```python
from build123d import *

# Parameters (mm, degrees)
SKETCH_1_W          = 48
SKETCH_1_H          = 30
EXTRUDE_1_DEPTH     = 30
SKETCH_2_W          = 28
SKETCH_2_H          = 15
CUT_EXTRUDE_1_DEPTH = 20
SKETCH_3_R          = 2.2
CUT_EXTRUDE_2_DEPTH = 20
SKETCH_4_R          = 2.5
CUT_EXTRUDE_3_DEPTH = 30
CUT_EXTRUDE_START   = -30
SKETCH_8_W          = 48
SKETCH_8_H          = 7
CUT_EXTRUDE_5_DEPTH = 30


with BuildPart() as part:
    # 草图1 → 凸台-拉伸1 (new body)
    with BuildSketch(Plane.XY):
        with Locations((-0.545454545, 1.527272727)):
            Rectangle(SKETCH_1_W, SKETCH_1_H)
    extrude(amount=EXTRUDE_1_DEPTH)

    # 草图2 → 切除-拉伸1 (cut)
    with BuildSketch(Plane(origin=(0, 0, 0), x_dir=(-1, 0, 0), z_dir=(0, 0, -1))):
        with Locations((0.545454545, -5.972727273)):
            Rectangle(SKETCH_2_W, SKETCH_2_H)
    extrude(amount=-CUT_EXTRUDE_1_DEPTH, mode=Mode.SUBTRACT)

    # 草图3 → 切除-拉伸2 (cut)
    with BuildSketch(Plane(origin=(0, 0, 20), x_dir=(-1, 0, 0), z_dir=(0, 0, -1))):
        with Locations((-10.454545455, -3.472727273)):
            Circle(SKETCH_3_R)
        with Locations((11.545454545, -3.472727273)):
            Circle(SKETCH_3_R)
    extrude(amount=-CUT_EXTRUDE_2_DEPTH, mode=Mode.SUBTRACT)

    # 草图4 → 切除-拉伸3 (cut)
    with BuildSketch(Plane.XZ.offset(13.472727273)):
        with Locations(Location((-19.545454545, 5, 0), (0, 0, 270))):
            Circle(SKETCH_4_R)
        with Locations(Location((-19.545454545, 23, 0), (0, 0, 270))):
            Circle(SKETCH_4_R)
        with Locations(Location((18.454545455, 23, 0), (0, 0, 270))):
            Circle(SKETCH_4_R)
        with Locations(Location((18.454545455, 5, 0), (0, 0, 270))):
            Circle(SKETCH_4_R)
    extrude(amount=-CUT_EXTRUDE_3_DEPTH, mode=Mode.SUBTRACT)

    # 草图8 → 切除-拉伸5 (cut)
    with BuildSketch(Plane.XY.offset(30).offset(CUT_EXTRUDE_START)):
        with Locations((-0.545454545, 13.027272727)):
            Rectangle(SKETCH_8_W, SKETCH_8_H)
    extrude(amount=CUT_EXTRUDE_5_DEPTH, mode=Mode.SUBTRACT)


solid = part.part
```
The listing builds one solid part. Answer for the finished solid, in the listing's coordinates (mm). A direction names the side the tool comes from. Round coordinates to 2 decimals unless told otherwise and drop trailing zeros. Write each loop counter-clockwise with the first axis right and the second up, starting at its lowest first coordinate (ties: lowest second). Pieces come first, ordered by that corner, then holes. Notation, with made-up numbers: (49.5, 19) -> (96.5, 19) arc R28 ccw to (96.5, 42) -> close; hole circle Ø2 at (-40, 85). An arc over 180 degrees is marked (long way). Answer as a JSON object with one key per item and string values. Group by question number.
Q1. Determine the mould class of faces 1 (the face through (-21.07, -2.13, 24.98)), 2 (the face through (-14.545, -6, 10)), 3 (the face through (-1, 3, 0)), 4 (the face through (-1, -2, 30)) for opening direction Z: pulls with the +Z half, pulls with the -Z half, needs draft (parallel to the pull), parting line crosses it, or undercut.
Q2. Which of the six approach directions +Z, -Z, +X, -X, +Y, -Y give full straight-line access (tool end or side, diameter ignored) to faces 5 (the face through (-21.763, -2.134, 3.846)), 6 (the face through (0, 1.527, 10))?
Q3. Section B-B (z = 24.75) is taken. Write down the section's boundary in (x, y).
Q4. Straight lines are drawn through the part: line 1 along X through (y, z) = (4.25, 23); line 2 along X through (y, z) = (2, 5.25); line 3 along X through (y, z) = (-6.25, 15.75). For each, find the intervals that lie inside material, in ascending order.
Q5. Each of these flat-tipped pins is pushed along its axis until it touches: pin 1 Ø8 at (x, z) = (18.45, 5) entering from -Y; pin 2 Ø2.5 at (x, y) = (10.45, -3.47) entering from +Z; pin 3 Ø1.5 at (x, z) = (7, 10) entering from -Y; pin 4 Ø2 at (x, y) = (-2.5, -3) entering from -Z. Where does it stop, or does it pass through?
Q6. Section D-D (x = -1.5) is taken. Write down the section's boundary in (y, z), plus the area to 3 significant figures.
Q7. Section A-A (z = 5) is taken. Write down the section's boundary in (x, y), plus the area to 3 significant figures.
Q8. Section C-C (y = -11) is taken. Write down the section's boundary in (x, z), plus the area to 3 significant figures.
Check values:
{
 "1": {"face 1": "undercut", "face 2": "needs draft", "face 3": "pulls with the -Z half", "face 4": "pulls with the +Z half"},
 "2": {"face 5": "+Y, -Y", "face 6": "-Z, -Y"},
 "3": {"outline": "(-24.55, -13.47) -> (-21.33, -13.47) -> (-21.33, 9.53) -> (-24.55, 9.53) -> close; (-17.76, -13.47) -> (16.67, -13.47) -> (16.67, 9.53) -> (-17.76, 9.53) -> close; (20.24, -13.47) -> (23.45, -13.47) -> (23.45, 9.53) -> (20.24, 9.53) -> close; hole circle Ø4.4 at (-11.55, -3.47); hole circle Ø4.4 at (10.45, -3.47)"},
 "4": {"line 1": "-24.55 to -22.05, -17.05 to 15.95, 20.95 to 23.45", "line 2": "-24.55 to -22.03, -17.06 to 15.97, 20.94 to 23.45", "line 3": "-24.55 to -14.55, 13.45 to 23.45"},
 "5": {"pin 1": "y = -13.47", "pin 2": "through", "pin 3": "y = 1.53", "pin 4": "z = 20"},
 "6": {"outline": "(-13.47, 20) -> (1.53, 20) -> (1.53, 0) -> (9.53, 0) -> (9.53, 30) -> (-13.47, 30) -> close", "area": "390 mm^2"},
 "7": {"outline": "(-24.55, -13.47) -> (-22.05, -13.47) -> (-22.05, 9.53) -> (-24.55, 9.53) -> close; (-17.05, -13.47) -> (-14.55, -13.47) -> (-14.55, 1.53) -> (13.45, 1.53) -> (13.45, -13.47) -> (15.95, -13.47) -> (15.95, 9.53) -> (-17.05, 9.53) -> close; (20.95, -13.47) -> (23.45, -13.47) -> (23.45, 9.53) -> (20.95, 9.53) -> close", "area": "454 mm^2"},
 "8": {"outline": "(-24.55, 0) -> (-14.55, 0) -> (-14.55, 20) -> (13.45, 20) -> (13.45, 0) -> (23.45, 0) -> (23.45, 30) -> (-24.55, 30) -> close; hole circle Ø5 at (-19.55, 5); hole circle Ø5 at (-19.55, 23); hole circle Ø5 at (18.45, 5); hole circle Ø5 at (18.45, 23)", "area": "801 mm^2"}
}
